```python
from build123d import *

# Parameters (mm, degrees)
SKETCH1_W           = 34.925
SKETCH1_H           = 19.05
SKETCH1_R           = 3.9624
BOSS_EXTRUDE1_DEPTH = 6.35


with BuildPart() as part:
    # Sketch1 → Boss-Extrude1 (new body)
    with BuildSketch(Plane.XY):
        with Locations((17.4625, 9.525)):
            Rectangle(SKETCH1_W, SKETCH1_H)
        with Locations((9.525, 9.525)):
            Circle(SKETCH1_R, mode=Mode.SUBTRACT)
    extrude(amount=BOSS_EXTRUDE1_DEPTH)


solid = part.part
```
Verification items for the finished model (mm, model axes). Coordinates: 2 decimals unless noted, no trailing zeros. Order: outer loops, then holes, each group sorted by start corner. A loop starts at its lowest first (then second) coordinate and runs counter-clockwise, first axis right, second up. Notation, with made-up numbers: (68.25, 78.5) - (74.25, 78.5) arc R31 cw to (74.25, 104.5) - close; hole circle Ø2 at (-21.75, 16.25). An arc over 180 degrees is marked (long way). Return JSON: item names as keys, results as strings.
(1) Go/stop test with a flat-tipped pin: pin 1 (6.5 mm diameter, centred on x = 9.525, y = 9.525, fed in from +Z). Record where the tip stops, or that it passes through.
Filled sheet:
{"pin 1": "passes through"}
(2) Mould release check, pull along X, two halves, no side actions. Record for faces 1 (the flat face through (0, 9, 3)), 2 (the flat face through (34.925, 9, 3)), 3 (the cylindrical face through (13.304, 10.715, 3.131)): pulls with the +X half, pulls with the -X half, needs draft (parallel to the pull), parting line crosses it, or undercut.
Filled sheet:
{"face 1": "pulls with the -X half", "face 2": "pulls with the +X half", "face 3": "undercut"}
(3) Section check C-C, the plane z = 4.5. Record the cut outline in (x, y) (3 decimals), and give its area (3 significant figures).
Filled sheet:
{"outline": "(0, 0) - (34.925, 0) - (34.925, 19.05) - (0, 19.05) - close; hole circle Ø7.925 at (9.525, 9.525)", "area": "616 mm^2"}
(4) Section check A-A, the plane y = 7. Record the cut outline in (x, z) (3 decimals), and give its area (3 significant figures).
Filled sheet:
{"outline": "(0, 0) - (6.471, 0) - (6.471, 6.35) - (0, 6.35) - close; (12.579, 0) - (34.925, 0) - (34.925, 6.35) - (12.579, 6.35) - close", "area": "183 mm^2"}
(5) Section check B-B, the plane x = 8.5. Record the cut outline in (y, z).
Filled sheet:
{"outline": "(0, 0) - (5.7, 0) - (5.7, 6.35) - (0, 6.35) - close; (13.35, 0) - (19.05, 0) - (19.05, 6.35) - (13.35, 6.35) - close"}
(6) Thickness scan on line 1 along Y through (x, z) = (9.5, 2.5); line 2 along X through (y, z) = (12.75, 0.75) (3 decimals); line 3 along Y through (x, z) = (8.5, 5.5). Record the ranges inside material, lowest first.
Filled sheet:
{"line 1": "y = 0 to 5.56, 13.49 to 19.05", "line 2": "x = 0 to 7.223, 11.827 to 34.925", "line 3": "y = 0 to 5.7, 13.35 to 19.05"}
